Here's how the part is built. I have some questions about the finished solid (model axes, mm). Face numbers are marked on the shaded views. A direction names the side the tool comes from. Give positions to 0.01 mm unless a question says otherwise; leave off trailing zeros. Loops run counter-clockwise (first coordinate to the right, second up) from the corner with the lowest first, then second, coordinate; pieces in that order, holes last.
Q1. For the marked faces 1, 2, 3 and 4, which set-ups out of +Z, -Z, +X, -X, +Y, -Y let a thin tool reach every point of the face, with its end or its side?
Q2. If we section it at C-C (z = 26.5): Please give me the cut outline in (x, y), plus the area to 3 significant figures.
Q3. If we section it at A-A (z = 14): Please give me the cut outline in (x, y).
Q4. If we section it at D-D (y = -22.5): Please give me the cut outline in (x, z), plus the area to 3 significant figures.
Q5. If we section it at B-B (x = 54): Please give me the cut outline in (y, z), plus the area to 3 significant figures.
Q6. We'd pull the mould along Y, two halves only. Please class the marked faces 5, 6, 7 and 8: +Y half, -Y half, draft (parallel to the pull), parting line (faces both ways), or undercut.
Q7. Will these pins go through, and if not, where does the flat tip stop? P1, Ø1, axis at y = 15.5, z = 24, coming from the +X side; P2, Ø2, axis at x = -11.5, z = 9, coming from the +Y side; P3, Ø9.5, axis at y = -49, z = 13, coming from the +X side.
Q8. I need wall thicknesses on line 1 (Z direction, x = -22, y = -15); line 2 (X direction, y = 0.5, z = 4); line 3 (X direction, y = -49, z = 22). Which ranges of each line are inside material? Lowest first, please.
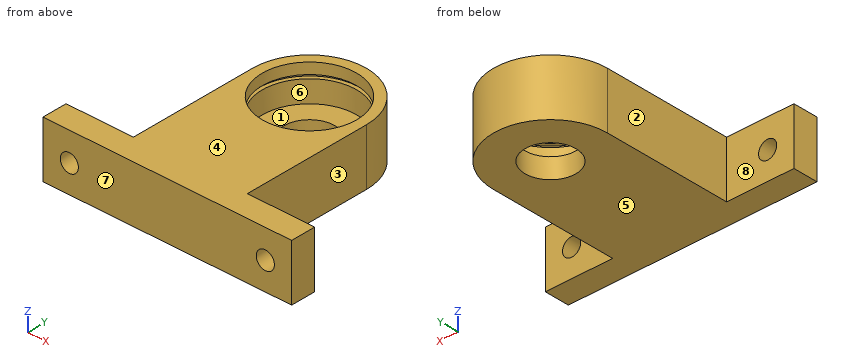
from build123d import *

# Parameters (mm, degrees)
SKETCH1_R           = 31.396947085
SKETCH1_R_2         = 12.5
BOSS_EXTRUDE1_DEPTH = 31
SKETCH2_R           = 5
CUT_EXTRUDE1_DEPTH  = 31
SKETCH3_R           = 14
CUT_EXTRUDE2_DEPTH  = 114.19357359
SKETCH5_R           = 26
CUT_EXTRUDE4_DEPTH  = 20
SKETCH6_R           = 28.1
CUT_EXTRUDE5_DEPTH  = 2


with BuildPart() as part:
    # Sketch1 → Boss-Extrude1 (new body)
    # profile 1 of 2: a face of its own
    with BuildSketch(Plane.XY):
        Circle(SKETCH1_R)
        with Locations(Location((0, 0, 0), (0, 0, 180))):
            Circle(SKETCH1_R_2, mode=Mode.SUBTRACT)
    # profile 2 of 2: a face of its own
    with BuildSketch(Plane.XY):
        with BuildLine():
            ThreePointArc((31.396947085, 0), (0, -31.396947085), (-31.396947085, 0))
            Line((-31.396947085, 0), (-31.396947085, -70.888581066))
            Line((-31.396947085, -70.888581066), (-68.506708087, -70.888581066))
            Line((-68.506708087, -70.888581066), (-68.506708087, -84.608605054))
            Line((-68.506708087, -84.608605054), (68.506708087, -84.608605054))
            Line((68.506708087, -84.608605054), (68.506708087, -70.888581066))
            Line((68.506708087, -70.888581066), (31.396947085, -70.888581066))
            Line((31.396947085, -70.888581066), (31.396947085, 0))
        make_face()
    extrude(amount=BOSS_EXTRUDE1_DEPTH)

    # Sketch2 → Cut-Extrude1 (cut)
    with BuildSketch(Plane(origin=(0, -70.888581066, 0), x_dir=(1, 0, 0), z_dir=(0, 1, 0))):
        with Locations(Location((54, -15.251041139, 0), (0, 0, 270))):
            Circle(SKETCH2_R)
        with Locations(Location((-54, -15.251041139, 0), (0, 0, 270))):
            Circle(SKETCH2_R)
    extrude(amount=-CUT_EXTRUDE1_DEPTH, mode=Mode.SUBTRACT)

    # Sketch3 → Cut-Extrude2 (cut, through all)
    with BuildSketch(Plane(origin=(0, 0, 0), x_dir=(-1, 0, 0), z_dir=(0, 0, -1))):
        Circle(SKETCH3_R)
    extrude(amount=-CUT_EXTRUDE2_DEPTH, mode=Mode.SUBTRACT)

    # Sketch5 → Cut-Extrude4 (cut)
    with BuildSketch(Plane.XY.offset(31)):
        Circle(SKETCH5_R)
    extrude(amount=-CUT_EXTRUDE4_DEPTH, mode=Mode.SUBTRACT)

    # Sketch6 → Cut-Extrude5 (cut)
    with BuildSketch(Plane.XY.offset(23)):
        Circle(SKETCH6_R)
    extrude(amount=CUT_EXTRUDE5_DEPTH, mode=Mode.SUBTRACT)


solid = part.part
Check sheet entries:
1. face 1: +Z
1. face 2: +Z, -Z, -X, +Y
1. face 3: +Z, -Z, +X, +Y
1. face 4: +Z, +X, -X, +Y, -Y
2. outline: (-68.51, -84.61) - (68.51, -84.61) - (68.51, -70.89) - (31.4, -70.89) - (31.4, 0) arc R31.4 ccw to (-31.4, 0) - (-31.4, -70.89) - (-68.51, -70.89) - close; hole circle Ø52 at (0, 0)
2. area: 5,760 mm2
3. outline: (-68.51, -84.61) - (-58.84, -84.61) - (-58.84, -70.89) - (-68.51, -70.89) - close; (-49.16, -84.61) - (49.16, -84.61) - (49.16, -70.89) - (31.4, -70.89) - (31.4, 0) arc R31.4 ccw to (-31.4, 0) - (-31.4, -70.89) - (-49.16, -70.89) - close; (58.84, -84.61) - (68.51, -84.61) - (68.51, -70.89) - (58.84, -70.89) - close; hole circle Ø52 at (0, 0)
4. outline: (-31.4, 0) - (31.4, 0) - (31.4, 31) - (13.03, 31) - (13.03, 25) - (16.83, 25) - (16.83, 23) - (13.03, 23) - (13.03, 11) - (-13.03, 11) - (-13.03, 23) - (-16.83, 23) - (-16.83, 25) - (-13.03, 25) - (-13.03, 31) - (-31.4, 31) - close
4. area: 1,410 mm2
5. outline: (-84.61, 0) - (-70.89, 0) - (-70.89, 10.25) - (-84.61, 10.25) - close; (-84.61, 20.25) - (-70.89, 20.25) - (-70.89, 31) - (-84.61, 31) - close
5. area: 288 mm2
6. face 5: draft
6. face 6: undercut
6. face 7: -Y half
6. face 8: +Y half
7. P1: stops at x = 27.58
7. P2: stops at y = 29.59
7. P3: stops at x = 31.4
8. line 1: z = 0 to 23, 25 to 31
8. line 2: x = -31.39 to -13.99, 13.99 to 31.39
8. line 3: x = -31.4 to 31.4
